```python
from build123d import *

# Parameters (mm, degrees)
BOSS_EXTRUDE1_DEPTH = 12


with BuildPart() as part:
    # Sketch1 → Boss-Extrude1 (new body)
    with BuildSketch(Plane.XY):
        with BuildLine():
            Line((0, 0), (420, 0))
            Line((420, 0), (446.084814008, 164.693033951))
            ThreePointArc((446.084814008, 164.693033951), (456.232022776, 182.812178968), (475.715464226, 190))
            Line((475.715464226, 190), (764.284535774, 190))
            ThreePointArc((764.284535774, 190), (783.767977224, 182.812178968), (793.915185992, 164.693033951))
            Line((793.915185992, 164.693033951), (820, 0))
            Line((820, 0), (1240, 0))
            Line((1240, 0), (1240, 208))
            Line((1240, 208), (1230, 208))
            Line((1230, 208), (1230, 268))
            Line((1230, 268), (850, 268))
            Line((850, 268), (850, 208))
            Line((850, 208), (830, 208))
            Line((830, 208), (830, 268))
            Line((830, 268), (410, 268))
            Line((410, 268), (410, 208))
            Line((410, 208), (390, 208))
            Line((390, 208), (390, 268))
            Line((390, 268), (10, 268))
            Line((10, 268), (10, 208))
            Line((10, 208), (0, 208))
            Line((0, 208), (0, 0))
        make_face()
    extrude(amount=BOSS_EXTRUDE1_DEPTH)


solid = part.part
```
Verification items for the finished model (mm, model axes). A direction names the side the tool comes from. Round coordinates to 2 decimals unless told otherwise and drop trailing zeros. Order: outer loops, then holes, each group sorted by start corner. A loop starts at its lowest first (then second) coordinate and runs counter-clockwise, first axis right, second up. Notation, with made-up numbers: (6, 51) - (23, 51) arc R18 cw to (23, 56) - close; hole circle Ø9 at (84, 74.5). An arc over 180 degrees is marked (long way). Use CSV: the item, a comma, the result in double quotes. Start each with the question number.
1) Go/stop test with flat-tipped pins: P1, Ø6, axis at y = 214, z = 3.5, coming from the -X side; P2, Ø3.5, axis at x = 396, z = 6, coming from the +Y side. Record where each tip stops, or that it passes through.
2) Section check C-C, the plane x = 512.5. Record the cut outline in (y, z).
3) Section check D-D, the plane y = 86.5. Record the cut outline in (x, z).
4) Section check A-A, the plane z = 9. Record the cut outline in (x, y), plus the area to 3 significant figures.
5) Access from +Z, -Z, +X, -X, +Y, -Y to the whole of each face (thin tool, end or side, straight path). Record for faces 3 (the flat face through (611, 195, 0)), 4 (the flat face through (432.86, 81.19, 5.92)).
6) Section check B-B, the plane y = 153. Record the cut outline in (x, z).
7) Mould release check, pull along X, two halves, no side actions. Record for faces 1 (the cylindrical face through (456.01, 182.62, 5.92)), 2 (the flat face through (611, 195, 12)): +X half, -X half, draft (parallel to the pull), parting line (faces both ways), or undercut.
8) Thickness scan on L1, parallel to X at y = 221.5, z = 8.25; L2, parallel to X at y = 143, z = 7.75; L3, parallel to X at y = 106, z = 9.5. Record the ranges inside material, lowest first.
Answers:
1,P1,"stops at x = 10"
1,P2,"stops at y = 208"
2,outline,"(190, 0) - (268, 0) - (268, 12) - (190, 12) - close"
3,outline,"(0, 0) - (433.7, 0) - (433.7, 12) - (0, 12) - close; (806.3, 0) - (1240, 0) - (1240, 12) - (806.3, 12) - close"
4,outline,"(0, 0) - (420, 0) - (446.08, 164.69) arc R30 cw to (475.72, 190) - (764.28, 190) arc R30 cw to (793.92, 164.69) - (820, 0) - (1240, 0) - (1240, 208) - (1230, 208) - (1230, 268) - (850, 268) - (850, 208) - (830, 208) - (830, 268) - (410, 268) - (410, 208) - (390, 208) - (390, 268) - (10, 268) - (10, 208) - (0, 208) - close"
4,area,"259,000 mm²"
5,face 3,"-Z, +X, -X, +Y, -Y"
5,face 4,"+Z, -Z, -Y"
6,outline,"(0, 0) - (444.23, 0) - (444.23, 12) - (0, 12) - close; (795.77, 0) - (1240, 0) - (1240, 12) - (795.77, 12) - close"
7,face 1,"undercut"
7,face 2,"draft"
8,L1,"x = 10 to 390, 410 to 830, 850 to 1230"
8,L2,"x = 0 to 442.65, 797.35 to 1240"
8,L3,"x = 0 to 436.79, 803.21 to 1240"
